Geometry: final body of the model. Coordinates: model frame, mm. Round coordinates to 2 decimals unless told otherwise and drop trailing zeros. Write each loop counter-clockwise with the first axis right and the second up, starting at its lowest first coordinate (ties: lowest second). Pieces come first, ordered by that corner, then holes. Notation, with made-up numbers: M -34,10 L -6,10 A5 cw -6,18 Z; hole C -4.75,22 d1. An arc over 180 degrees is marked long. Put each result on its own line as item: value. Start each with the question number.
```python
from build123d import *

# Parameters (mm, degrees)
SKETCH_1_R          = 9
EXTRUDE_1_DEPTH     = 10
FILLET_1_R          = 10
SKETCH_2_R          = 9
CUT_EXTRUDE_1_DEPTH = 279.025277116


with BuildPart() as part:
    # 草图1 → 凸台-拉伸1 (new body)
    with BuildSketch(Plane.XY):
        with BuildLine():
            Line((-67.5, 116.913429511), (-125, 216.506350946))
            ThreePointArc((-125, 216.506350946), (0, 250), (125, 216.506350946))
            Line((125, 216.506350946), (67.5, 116.913429511))
            ThreePointArc((67.5, 116.913429511), (0, 135), (-67.5, 116.913429511))
        make_face()
        with Locations((0, 155)):
            Circle(SKETCH_1_R, mode=Mode.SUBTRACT)
        with Locations((59.315932017, 143.201327539)):
            Circle(SKETCH_1_R, mode=Mode.SUBTRACT)
        with Locations((-59.315932017, 143.201327539)):
            Circle(SKETCH_1_R, mode=Mode.SUBTRACT)
    extrude(amount=EXTRUDE_1_DEPTH)

    # 圆角1
    fillet_1_edges = [part.edges().sort_by_distance(p)[0] for p in [
        (-67.5, 116.913429511, 5),
        (-125, 216.506350946, 5),
        (125, 216.506350946, 5),
        (67.5, 116.913429511, 5),
    ]]
    fillet(fillet_1_edges, radius=FILLET_1_R)

    # 草图2 → 切除-拉伸1 (cut, through all)
    with BuildSketch(Plane.XY.offset(10)):
        with Locations((0, 230)):
            Circle(SKETCH_2_R)
        with Locations((88.017189444, 212.492292478)):
            Circle(SKETCH_2_R)
        with Locations(Location((-88.017189444, 212.492292478, 0), (0, 0, 180))):
            Circle(SKETCH_2_R)
    extrude(amount=-CUT_EXTRUDE_1_DEPTH, mode=Mode.SUBTRACT)


solid = part.part
```
1) Section C-C, the plane x = -61.5. Output: boundary loops of the cut face in (y, z).
2) Section B-B, the plane y = 230. Output: boundary loops of the cut face in (x, z).
3) Section D-D, the plane z = 2.25. Output: boundary loops of the cut face in (x, y).
4) Draft query along Y for faces 1 (the face through (-1.687, 249.994, 4.93)), 2 (the face through (66.49, 120.68, 5.07)), 3 (the face through (-1.172, 238.923, 5.07)). Return one class per face: +Y half, -Y half, draft (parallel to the pull), parting line (faces both ways), or undercut.
5) First-contact query: pin 1 (1 mm diameter, centred on x = -58, z = 1, fed in from +Y); pin 2 (4 mm diameter, centred on y = 179, z = 5, fed in from -X); pin 3 (1.5 mm diameter, centred on x = -84, z = 5.5, fed in from -Y). Flat tips, straight axial feed; report the tip coordinate or a pass-through.
6) Section A-A, the plane x = 0. Output: boundary loops of the cut face in (y, z).
7) Ray query, probe 1 along X at (y, z) = (207, 2.25); probe 2 along X at (y, z) = (204.5, 3.25); probe 3 along Y at (x, z) = (-58, 3). Return the intervals inside material, ascending.
Solved:
1. outline: M 120.51,0 L 134.47,0 L 134.47,10 L 120.51,10 Z; M 151.93,0 L 242.32,0 L 242.32,10 L 151.93,10 Z
2. outline: M -97.98,0 L -9,0 L -9,10 L -97.98,10 Z; M 9,0 L 97.98,0 L 97.98,10 L 9,10 Z
3. outline: M -119.9,207.67 L -72.33,125.27 A10 ccw -59.28,121.29 A135 cw 59.28,121.29 A10 ccw 72.33,125.27 L 119.9,207.67 A10 ccw 115.87,221.53 A250 ccw -115.87,221.53 A10 ccw Z; hole C -88.02,212.49 d18; hole C -59.32,143.2 d18; hole C 0,155 d18; hole C 0,230 d18; hole C 59.32,143.2 d18; hole C 88.02,212.49 d18
4. face 1: +Y half
4. face 2: -Y half
4. face 3: undercut
5. pin 1: stops at y = 243.3
5. pin 2: stops at x = -104.5
5. pin 3: stops at y = 144.19
6. outline: M 135,0 L 146,0 L 146,10 L 135,10 Z; M 164,0 L 221,0 L 221,10 L 164,10 Z; M 239,0 L 250,0 L 250,10 L 239,10 Z
7. probe 1: x = -119.51 to -95.15, -80.89 to 80.89, 95.15 to 119.51
7. probe 2: x = -118.07 to -92.16, -83.88 to 83.88, 92.16 to 118.07
7. probe 3: y = 121.91 to 134.3, 152.1 to 243.18
